For this review, take the finished solid that the model builds, in its own axes (mm). Give positions to 0.01 mm unless a question says otherwise; leave off trailing zeros. Write each loop counter-clockwise with the first axis right and the second up, starting at its lowest first coordinate (ties: lowest second). Pieces come first, ordered by that corner, then holes.
1) For P1, Ø5, axis at x = 0, z = 0, coming from the +Y side; P2, Ø0.5, axis at x = -56.5, y = 0.5, coming from the +Z side, all flat-tipped, find the tip position at first contact; note any pin that passes through.
2) Draft analysis for pull direction X (two halves, no side actions). For faces 1 (the face through (-1.952, 0.493, -0.434)), 2 (the face through (1, 0, 17)), 3 (the face through (-80.54, 0.49, -17.88)), state which applies: pulls with the +X half, pulls with the -X half, needs draft (parallel to the pull), parting line crosses it, or undercut.
3) We need section C-C on x = 70. Give the boundary of the cut face in (y, z), and give its area (3 significant figures).
4) Wall thickness on line 1 along X through (y, z) = (0.3, 0); line 2 along X through (y, z) = (0.45, -0.5); line 3 along X through (y, z) = (0.25, 33): over which ranges is each line inside the solid? List them lowest first.
5) We need section D-D on z = -56.5. Give the boundary of the cut face in (x, y).
6) We need section A-A on y = 0.3. Give the boundary of the cut face in (x, z), and give its area (3 significant figures).
7) We need section B-B on x = -52. Give the boundary of the cut face in (y, z), and give its area (3 significant figures).
from build123d import *

# Parameters (mm, degrees)
SKETCH1_R           = 82.5
SKETCH1_R_2         = 1.5
SKETCH1_R_3         = 2
SKETCH1_W           = 64.8
SKETCH1_H           = 8.3
BOSS_EXTRUDE1_DEPTH = 1


with BuildPart() as part:
    # Sketch1 → Boss-Extrude1 (new body)
    with BuildSketch(Plane(origin=(0, 0, 0), x_dir=(1, 0, 0), z_dir=(0, 1, 0))):
        with Locations(Location((0, 0, 0), (0, 0, 270))):
            Circle(SKETCH1_R)
        with Locations(Location((-21.4, -21.4, 0), (0, 0, 270))):
            Circle(SKETCH1_R_2, mode=Mode.SUBTRACT)
        with Locations(Location((37.6, -33, 0), (0, 0, 270))):
            Circle(SKETCH1_R_2, mode=Mode.SUBTRACT)
        with Locations(Location((0, 0, 0), (0, 0, 270))):
            Circle(SKETCH1_R_3, mode=Mode.SUBTRACT)
        with Locations((-40.45, 0)):
            Rectangle(SKETCH1_W, SKETCH1_H, mode=Mode.SUBTRACT)
        with Locations((40.45, 0)):
            Rectangle(SKETCH1_W, SKETCH1_H, mode=Mode.SUBTRACT)
    extrude(amount=BOSS_EXTRUDE1_DEPTH)


solid = part.part
Results list:
1. P1: stops at y = 1
1. P2: stops at z = 60.35
2. face 1: undercut
2. face 2: needs draft
2. face 3: parting line crosses it
3. outline: (0, -43.66) - (1, -43.66) - (1, -4.15) - (0, -4.15) - close; (0, 4.15) - (1, 4.15) - (1, 43.66) - (0, 43.66) - close
3. area: 79.0 mm2
4. line 1: x = -82.5 to -72.85, -8.05 to -2, 2 to 8.05, 72.85 to 82.5
4. line 2: x = -82.5 to -72.85, -8.05 to -1.94, 1.94 to 8.05, 72.85 to 82.5
4. line 3: x = -75.61 to 36.1, 39.1 to 75.61
5. outline: (-60.12, 0) - (60.12, 0) - (60.12, 1) - (-60.12, 1) - close
6. outline: circle Ø165 at (0, 0); hole (-72.85, -4.15) - (-8.05, -4.15) - (-8.05, 4.15) - (-72.85, 4.15) - close; hole circle Ø3 at (-21.4, 21.4); hole circle Ø4 at (0, 0); hole (8.05, -4.15) - (72.85, -4.15) - (72.85, 4.15) - (8.05, 4.15) - close; hole circle Ø3 at (37.6, 33)
6. area: 20,300 mm2
7. outline: (0, -64.05) - (1, -64.05) - (1, -4.15) - (0, -4.15) - close; (0, 4.15) - (1, 4.15) - (1, 64.05) - (0, 64.05) - close
7. area: 120 mm2
